from build123d import *
from build123d.topology import SkipClean

# Parameters (mm, degrees)
SKETCH_1_R          = 3
EXTRUDE_1_DEPTH     = 100
EXTRUDE_3_DEPTH     = 5
EXTRUDE_START       = 5
EXTRUDE_4_DEPTH     = 5
SKETCH_9_R          = 1.5
CUT_EXTRUDE_1_DEPTH = 5
SKETCH_10_R         = 1.5
CUT_EXTRUDE_2_DEPTH = 5


with BuildPart() as part:
    # 草图1 → 凸台-拉伸1 (new body)
    with BuildSketch(Plane.XY):
        Circle(SKETCH_1_R)
    extrude(amount=EXTRUDE_1_DEPTH)

    # 草图2 → 凸台-拉伸3 (add)
    with SkipClean():  # the faces are left unmerged after this step: merging them gives an invalid solid
        with BuildSketch(Plane.XY.offset(100)):
            with BuildLine():
                Line((-2.891366459, 0.8), (2.891366459, 0.8))
                ThreePointArc((2.891366459, 0.8), (3, 0), (2.891366459, -0.8))
                Line((2.891366459, -0.8), (-2.891366459, -0.8))
                ThreePointArc((-2.891366459, -0.8), (-3, 0), (-2.891366459, 0.8))
            make_face()
        extrude(amount=EXTRUDE_3_DEPTH)

    # 草图8 → 凸台-拉伸4 (add)
    with SkipClean():  # the faces are left unmerged after this step: merging them gives an invalid solid
        with BuildSketch(Plane(origin=(0, 0, 0), x_dir=(-1, 0, 0), z_dir=(0, 0, -1)).offset(EXTRUDE_START)):
            with BuildLine():
                Line((-2.891366459, 0.8), (2.891366459, 0.8))
                ThreePointArc((2.891366459, 0.8), (3, 0), (2.891366459, -0.8))
                Line((2.891366459, -0.8), (-2.891366459, -0.8))
                ThreePointArc((-2.891366459, -0.8), (-3, 0), (-2.891366459, 0.8))
            make_face()
        extrude(amount=-EXTRUDE_4_DEPTH)

    # 草图9 → 切除-拉伸1 (cut)
    with SkipClean():  # the faces are left unmerged after this step: merging them gives an invalid solid
        with BuildSketch(Plane(origin=(0, 0.8, 0), x_dir=(1, 0, 0), z_dir=(0, 1, 0))):
            with Locations(Location((0, 2.5, 0), (0, 0, 270))):
                Circle(SKETCH_9_R)
        extrude(amount=-CUT_EXTRUDE_1_DEPTH, mode=Mode.SUBTRACT)

    # 草图10 → 切除-拉伸2 (cut)
    with SkipClean():  # the faces are left unmerged after this step: merging them gives an invalid solid
        with BuildSketch(Plane(origin=(0, 0.8, 0), x_dir=(1, 0, 0), z_dir=(0, 1, 0))):
            with Locations(Location((0, -102.5, 0), (0, 0, 270))):
                Circle(SKETCH_10_R)
        extrude(amount=-CUT_EXTRUDE_2_DEPTH, mode=Mode.SUBTRACT)


solid = part.part
Model file for the job. Use its own axes, mm. A direction names the side the tool comes from. Give positions to 0.01 mm unless a question says otherwise; leave off trailing zeros. Write each loop counter-clockwise with the first axis right and the second up, starting at its lowest first coordinate (ties: lowest second). Pieces come first, ordered by that corner, then holes. Notation, with made-up numbers: (-14.5, 81) -> (-2.5, 81) arc R31 ccw to (-2.5, 114) -> close; hole circle Ø4 at (-20, 30). An arc over 180 degrees is marked (long way). Write item = value, one per line.
(1) Mould opens along Z. For faces 1 (the face through (0, 0, 101)), 2 (the face through (0, -2, 100)), 3 (the face through (0, 2, 0)) say: released by +Z, released by -Z, zero draft, split by the parting line, or undercut.
Determined:
face_1 = undercut
face_2 = released by +Z
face_3 = released by -Z
(2) Flat gauge pins, fed straight in: P1, Ø0.7, axis at x = 0.5, y = -2, coming from the +Z side; P2, Ø1.5, axis at x = 0.5, z = 102.5, coming from the +Y side; P3, Ø0.7, axis at x = 0, y = 2, coming from the -Z side; P4, Ø1.5, axis at x = -1, z = -3, coming from the -Y side. Where does each tip first touch, or does it go through?
Determined:
P1 = 100
P2 = through
P3 = 0
P4 = -0.8
(3) Probe line 1 along X through (y, z) = (0.35, 102.5); line 2 along Z through (x, y) = (0.5, 0.6); line 3 along Z through (x, y) = (-2, 0.85). List the from-to ranges inside material, lowest first.
Determined:
line_1 = -2.98 to -1.5, 1.5 to 2.98
line_2 = -5 to -3.91, -1.09 to 101.09, 103.91 to 105
line_3 = 0 to 100
(4) Tool access for faces 4 (the face through (0, -0.8, -4.2)), 5 (the face through (0, 0.8, -4.2)), 6 (the face through (0, 2, 100)): list every direction of +Z, -Z, +X, -X, +Y, -Y with a clear straight run to the whole face (end or side of a thin tool).
Determined:
face_4 = -Z, +X, -X, -Y
face_5 = -Z, +X, -X, +Y
face_6 = +Z, +X, -X, +Y
(5) Slice it at C-C, the plane z = 64. Give the cut face in (x, y).
Determined:
outline = circle Ø6 at (0, 0)
(6) Slice it at A-A, the plane x = 0. Give the cut face in (y, z).
Determined:
outline = (-3, 0) -> (-0.8, 0) -> (-0.8, -1) -> (0.8, -1) -> (0.8, 0) -> (3, 0) -> (3, 100) -> (0.8, 100) -> (0.8, 101) -> (-0.8, 101) -> (-0.8, 100) -> (-3, 100) -> close; (-0.8, -5) -> (0.8, -5) -> (0.8, -4) -> (-0.8, -4) -> close; (-0.8, 104) -> (0.8, 104) -> (0.8, 105) -> (-0.8, 105) -> close
(7) Slice it at B-B, the plane z = 102.5. Give the cut face in (x, y).
Determined:
outline = (-2.89, -0.8) -> (-1.5, -0.8) -> (-1.5, 0.8) -> (-2.89, 0.8) arc R3 ccw to start; (1.5, -0.8) -> (2.89, -0.8) arc R3 ccw to (2.89, 0.8) -> (1.5, 0.8) -> close
